Here's how the part is built. I have some questions about the finished solid (model axes, mm). Face numbers are marked on the shaded views. A direction names the side the tool comes from. Coordinates: 2 decimals unless noted, no trailing zeros. Write each loop counter-clockwise with the first axis right and the second up, starting at its lowest first coordinate (ties: lowest second). Pieces come first, ordered by that corner, then holes. Notation, with made-up numbers: M 31,18.5 L 49,18.5 A29 ccw 49,53.5 Z; hole C 69,-36.75 d1. An arc over 180 degrees is marked long. Write each question's results on one line, items separated by ' | '. Start each with the question number.
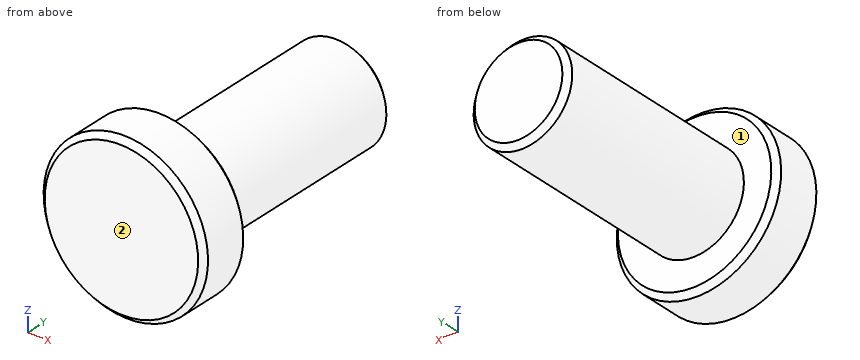
from build123d import *

# Parameters (mm, degrees)
CHAMFER1_SIZE = 0.5


with BuildPart() as part:
    # Sketch1 → Revolve1 (revolve)
    with BuildSketch(Plane(origin=(0, 0, 0), x_dir=(0, 0, -1), z_dir=(1, 0, 0))):
        Polygon((0, 25), (4.5, 25), (4.5, 5), (7.5, 5), (7.5, 0), (0, 0), align=None)
    revolve(axis=Axis((0, 0, 0), (0, 1, 0)))

    # Chamfer1
    chamfer1_edges = [part.edges().sort_by_distance(p)[0] for p in [
        (0, 0, 7.5),
        (0, 5, 7.5),
        (0, 25, 4.5),
    ]]
    chamfer(chamfer1_edges, length=CHAMFER1_SIZE)


solid = part.part
1) Please list where these lines run through material, in increasing order: line 1 (X direction, y = 14, z = 0); line 2 (Y direction, x = -3.5, z = 3.5); line 3 (Z direction, x = 3.75, y = 1.75). Write a range as [from, to].
2) I want a section at A-A, the plane x = 0. Write out the boundary of the cut face in (y, z), then the cut area to 3 significant figures.
3) For pin 1 Ø3 at (x, z) = (-4.5, 1.5) entering from +Y; pin 2 Ø3 at (x, y) = (-3.5, 10.5) entering from -Z, each with a flat end and sliding along its axis, tell me the tip position at first contact or that it passes through.
4) For the marked faces 1 and 2, which set-ups out of +Z, -Z, +X, -X, +Y, -Y let a thin tool reach every point of the face, with its end or its side?
5) I want a section at B-B, the plane z = 0. Write out the boundary of the cut face in (x, y), then the cut area to 3 significant figures.
6) I want a section at C-C, the plane y = 19.25. Write out the boundary of the cut face in (x, z), then the cut area to 3 significant figures.
Output:
1) line 1: x = [-4.5, 4.5] | line 2: y = [0, 5] | line 3: z = [-6.5, 6.5]
2) outline: M 0,-7 L 0.5,-7.5 L 4.5,-7.5 L 5,-7 L 5,-4.5 L 24.5,-4.5 L 25,-4 L 25,4 L 24.5,4.5 L 5,4.5 L 5,7 L 4.5,7.5 L 0.5,7.5 L 0,7 Z | area: 254 mm2
3) pin 1: stops at y = 25 | pin 2: stops at z = -4.03
4) face 1: +Y | face 2: +Z, -Z, +X, -X, -Y
5) outline: M -7.5,0.5 L -7,0 L 7,0 L 7.5,0.5 L 7.5,4.5 L 7,5 L 4.5,5 L 4.5,24.5 L 4,25 L -4,25 L -4.5,24.5 L -4.5,5 L -7,5 L -7.5,4.5 Z | area: 254 mm2
6) outline: C 0,0 d9 | area: 63.6 mm2
